```python
from build123d import *

# Parameters (mm, degrees)
BOSS_EXTRUDE1_DEPTH    = 30
M16_TAPPED_HOLE1_D     = 14
M16_TAPPED_HOLE1_DEPTH = 45
M16_TAPPED_HOLE1_TIP   = 4.206024333


with BuildPart() as part:
    # Sketch1 → Boss-Extrude1 (new body)
    with BuildSketch(Plane.XY):
        Polygon((0, 317), (200, 317), (200, 492), (2118, 492), (2118, 0), (0, 0), align=None)
    extrude(amount=BOSS_EXTRUDE1_DEPTH)

    # M16 Tapped Hole1
    with Locations(Plane(origin=(918, 492, 15), x_dir=(0, 0, 1), z_dir=(0, 1, 0))):
        with Locations((0, 0), (0, 100), (0, 1150), (0, 1050)):
            Hole(M16_TAPPED_HOLE1_D / 2, depth=M16_TAPPED_HOLE1_DEPTH)
            with Locations((0, 0, -(M16_TAPPED_HOLE1_DEPTH + M16_TAPPED_HOLE1_TIP / 2))):  # 118° drill point
                Cone(0, M16_TAPPED_HOLE1_D / 2, M16_TAPPED_HOLE1_TIP, mode=Mode.SUBTRACT)


solid = part.part
```
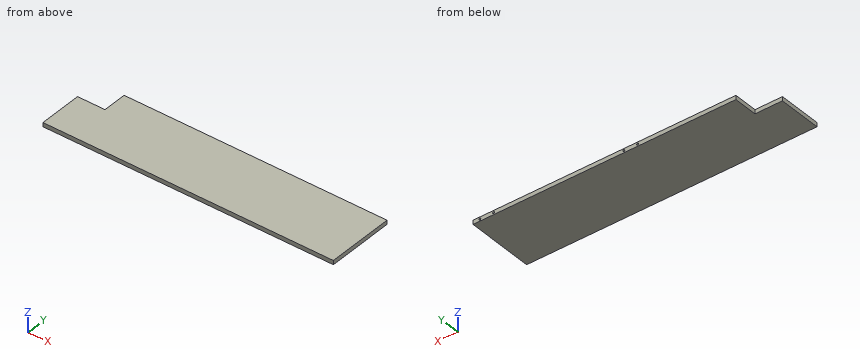
Geometry: final body of the model. Coordinates: model frame, mm. Round coordinates to 2 decimals unless told otherwise and drop trailing zeros. Order: outer loops, then holes, each group sorted by start corner. A loop starts at its lowest first (then second) coordinate and runs counter-clockwise, first axis right, second up. Notation, with made-up numbers: (61.5, 38) -> (119.5, 38) arc R27 cw to (119.5, 75) -> close; hole circle Ø7 at (-10, 65). An arc over 180 degrees is marked (long way). Use one line per item in the form item = value. Start each with the question number.
1. Line query: probe 1 along X at (y, z) = (463, 15); probe 2 along Z at (x, y) = (2068, 465.5); probe 3 along X at (y, z) = (435, 2.5). Output: solid intervals per line, ascending.
2. Cut plane A-A (y = 347.5). Return the cut outline in (x, z), then the cut area to 3 significant figures.
3. Pin query (flat end, axial travel): pin 1 Ø9 at (x, z) = (116, 9.5) entering from +Y. Return the tip coordinate at first contact, or that it passes through.
Solution:
q1.probe_1 = 200 to 911, 925 to 1011, 1025 to 1961, 1975 to 2061, 2075 to 2118
q1.probe_2 = 0 to 8, 22 to 30
q1.probe_3 = 200 to 2118
q2.outline = (200, 0) -> (2118, 0) -> (2118, 30) -> (200, 30) -> close
q2.area = 57,500 mm^2
q3.pin_1 = 317
